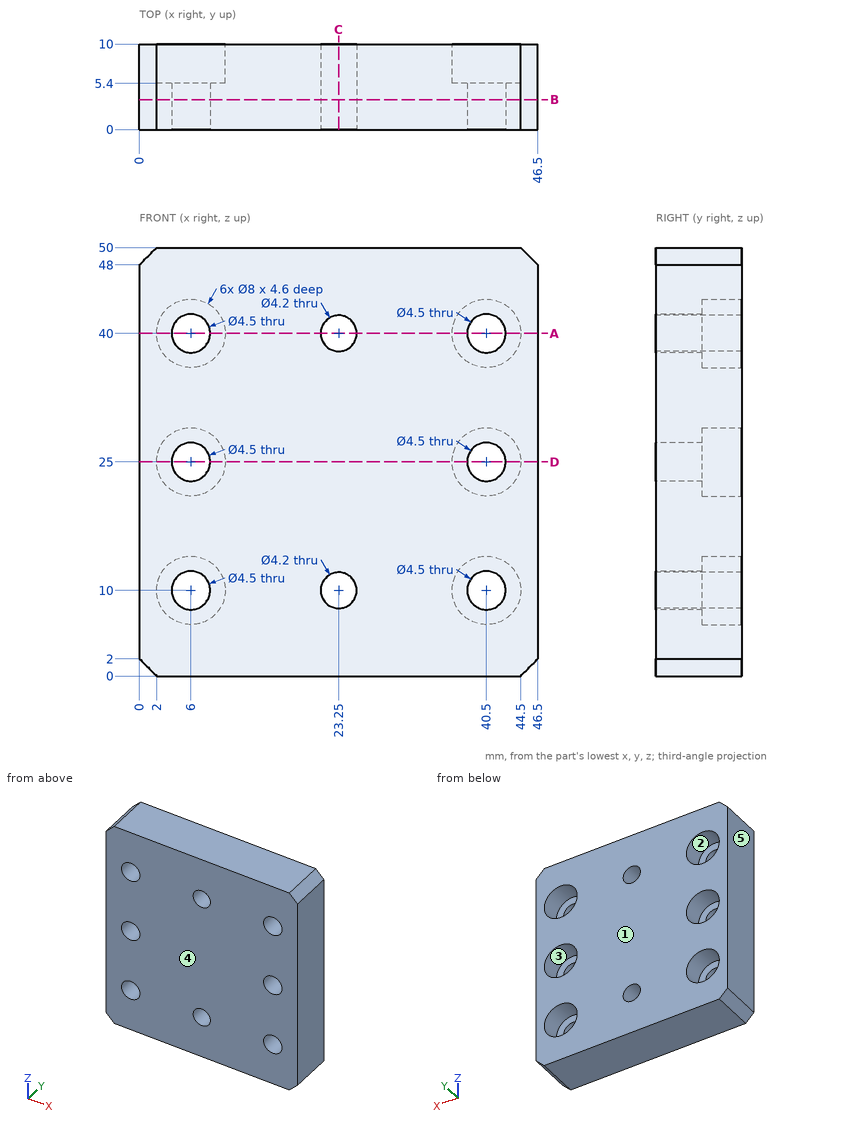
Input: dimensioned drawing with shaded views. Units: mm. Origin: part minimum x, y, z. A direction names the side the tool comes from. Round coordinates to 2 decimals unless told otherwise and drop trailing zeros. Order: outer loops, then holes, each group sorted by start corner. A loop starts at its lowest first (then second) coordinate and runs counter-clockwise, first axis right, second up.
Q1. Mould query, pull axis X, two halves, no side actions, for the marked faces 3, 4 and 5. Classes: released by +X, released by -X, zero draft, split by the parting line, or undercut.
Result sheet:
face 3: undercut
face 4: zero draft
face 5: released by -X
Q2. Section B-B, the plane y = 3.5. Give the number of separate pieces and of enclosed holes in the cut face, and give its area (3 significant figures).
Result sheet:
separate pieces: 1
enclosed holes: 8
area: 2,190 mm2
Q3. Section C-C, the plane x = 23.25. Output: boundary loops of the cut face in (y, z).
Result sheet:
outline: (0, 0) - (10, 0) - (10, 7.9) - (0, 7.9) - close; (0, 12.1) - (10, 12.1) - (10, 37.9) - (0, 37.9) - close; (0, 42.1) - (10, 42.1) - (10, 50) - (0, 50) - close
Q4. Section A-A, the plane z = 40. Output: boundary loops of the cut face in (x, y).
Result sheet:
outline: (0, 0) - (3.75, 0) - (3.75, 5.4) - (2, 5.4) - (2, 10) - (0, 10) - close; (8.25, 0) - (21.15, 0) - (21.15, 10) - (10, 10) - (10, 5.4) - (8.25, 5.4) - close; (25.35, 0) - (38.25, 0) - (38.25, 5.4) - (36.5, 5.4) - (36.5, 10) - (25.35, 10) - close; (42.75, 0) - (46.5, 0) - (46.5, 10) - (44.5, 10) - (44.5, 5.4) - (42.75, 5.4) - close
Q5. Material intervals for probe 1 along Z at (x, y) = (6, 7.3); probe 2 along X at (y, z) = (1.4, 40); probe 3 along Z at (x, y) = (6, 1.5), sorted ascending.
Result sheet:
probe 1: z = 0 to 6, 14 to 21, 29 to 36, 44 to 50
probe 2: x = 0 to 3.75, 8.25 to 21.15, 25.35 to 38.25, 42.75 to 46.5
probe 3: z = 0 to 7.75, 12.25 to 22.75, 27.25 to 37.75, 42.25 to 50
Q6. Pin query (flat end, axial travel): pin 1 (6 mm diameter, centred on x = 23, z = 11.5, fed in from +Y); pin 2 (6 mm diameter, centred on x = 6, z = 40, fed in from +Y). Return the tip coordinate at first contact, or that it passes through.
Result sheet:
pin 1: stops at y = 10
pin 2: stops at y = 5.4
Q7. Section D-D, the plane z = 25. Output: boundary loops of the cut face in (x, y), and give its area (3 significant figures).
Result sheet:
outline: (0, 0) - (3.75, 0) - (3.75, 5.4) - (2, 5.4) - (2, 10) - (0, 10) - close; (8.25, 0) - (38.25, 0) - (38.25, 5.4) - (36.5, 5.4) - (36.5, 10) - (10, 10) - (10, 5.4) - (8.25, 5.4) - close; (42.75, 0) - (46.5, 0) - (46.5, 10) - (44.5, 10) - (44.5, 5.4) - (42.75, 5.4) - close
area: 343 mm2
Q8. Access query for the marked faces 1 and 2. Directions: +Z, -Z, +X, -X, +Y, -Y. A direction counts if a zero-diameter tool reaches every point of the face in a straight line with its end or side. Return the directions, or none.
Result sheet:
face 1: +Z, -Z, +X, -X, +Y
face 2: +Y
